Verification items for this drawing (mm, ordinates from the low corner). Round coordinates to 2 decimals unless told otherwise and drop trailing zeros. Order: outer loops, then holes, each group sorted by start corner. A loop starts at its lowest first (then second) coordinate and runs counter-clockwise, first axis right, second up. Notation, with made-up numbers: (26.5, 1) -> (66.5, 1) arc R25 cw to (66.5, 40) -> close; hole circle Ø6 at (44, 74.5). An arc over 180 degrees is marked (long way). Answer in a Markdown table with one row per item.
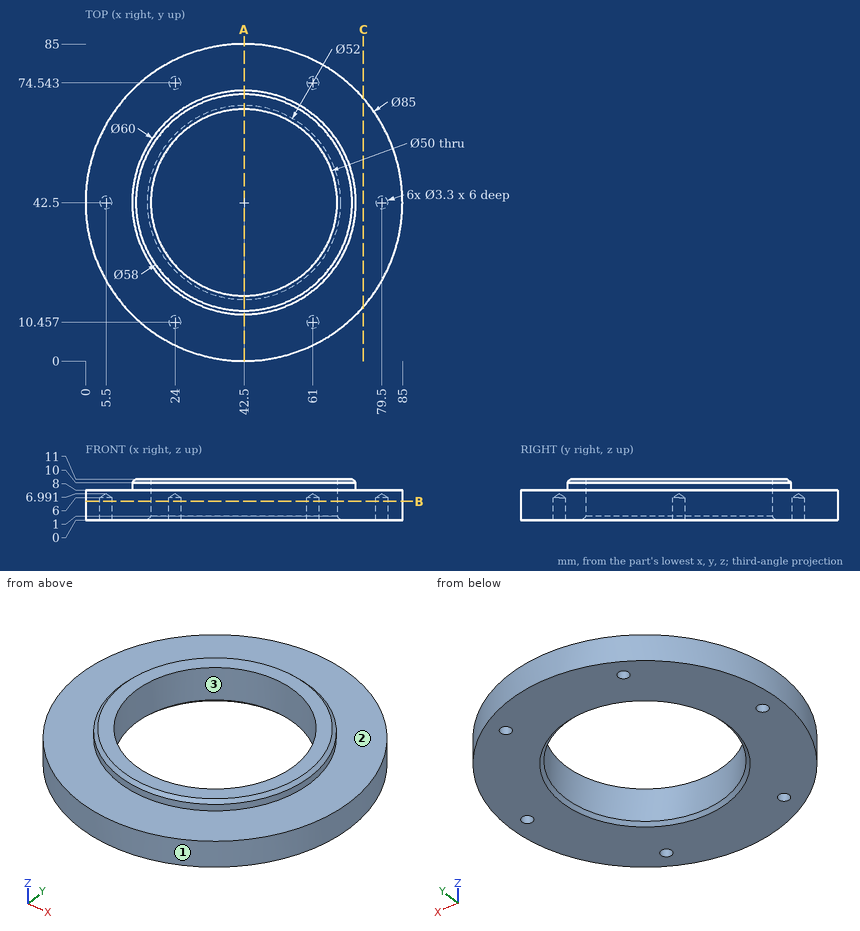
Item 1: Mould release check, pull along Y, two halves, no side actions. Record for the marked faces 1, 2 and 3: pulls with the +Y half, pulls with the -Y half, needs draft (parallel to the pull), parting line crosses it, or undercut.
Result sheet:
| item | result |
|---|---|
| face 1 | parting line crosses it |
| face 2 | needs draft |
| face 3 | undercut |
Item 2: Depth check by flat-ended pin: P1, Ø8, axis at x = 59, y = 51, coming from the +Z side; P2, Ø4.5, axis at x = 61, y = 74.54, coming from the +Z side; P3, Ø5, axis at x = 30.5, z = 7, coming from the -Y side (1 decimal); P4, Ø5, axis at x = 34, z = 8, coming from the +Y side. Enter the tip coordinate at first touch or a pass-through.
Result sheet:
| item | result |
|---|---|
| P1 | passes through |
| P2 | stops at z = 8 |
| P3 | stops at y = 1.1 |
| P4 | stops at y = 84.57 |
Item 3: Cross-section at A-A (x = 42.5). Record the boundary of the cut face in (y, z).
Result sheet:
| item | result |
|---|---|
| outline | (0, 0) -> (16.5, 0) -> (17.5, 1) -> (17.5, 11) -> (13.5, 11) -> (12.5, 10) -> (12.5, 8) -> (0, 8) -> close; (67.5, 1) -> (68.5, 0) -> (85, 0) -> (85, 8) -> (72.5, 8) -> (72.5, 10) -> (71.5, 11) -> (67.5, 11) -> close |
Item 4: Scan lines: line 1 (Y direction, x = 42.5, z = 7.75); line 2 (Y direction, x = 42.5, z = 8.75); line 3 (Z direction, x = 77, y = 48.5). Record each from-to range of solid material in increasing order. Write a range as [from, to].
Result sheet:
| item | result |
|---|---|
| line 1 | y = [0, 17.5], [67.5, 85] |
| line 2 | y = [12.5, 17.5], [67.5, 72.5] |
| line 3 | z = [0, 8] |
Item 5: Cross-section at B-B (z = 5). Record the boundary of the cut face in (x, y).
Result sheet:
| item | result |
|---|---|
| outline | circle Ø85 at (42.5, 42.5); hole circle Ø3.3 at (5.5, 42.5); hole circle Ø50 at (42.5, 42.5); hole circle Ø3.3 at (24, 10.46); hole circle Ø3.3 at (24, 74.54); hole circle Ø3.3 at (61, 10.46); hole circle Ø3.3 at (61, 74.54); hole circle Ø3.3 at (79.5, 42.5) |
Item 6: Cross-section at C-C (x = 74.5). Record the boundary of the cut face in (y, z).
Result sheet:
| item | result |
|---|---|
| outline | (14.53, 0) -> (70.47, 0) -> (70.47, 8) -> (14.53, 8) -> close |
